```python
from build123d import *

# Parameters (mm, degrees)
SKETCH1_W                                            = 4
SKETCH1_H                                            = 10
BOSS_EXTRUDE1_DEPTH                                  = 18
HOLE_SIZE_SLOTTED_COUNTERSUNK_WOOD_SCREW_D           = 2.4
HOLE_SIZE_SLOTTED_COUNTERSUNK_WOOD_SCREW_CSINK_D     = 4.5
HOLE_SIZE_SLOTTED_COUNTERSUNK_WOOD_SCREW_CSINK_ANGLE = 90
M2_TAPPED_HOLE1_D                                    = 1.6
M2_TAPPED_HOLE1_DEPTH                                = 6.4
M2_TAPPED_HOLE1_TIP                                  = 0.480688495
FILLET1_R                                            = 2.5
CHAMFER1_SIZE                                        = 0.2


with BuildPart() as part:
    # Sketch1 → Boss-Extrude1 (new body)
    with BuildSketch(Plane(origin=(0, 0, 0), x_dir=(1, 0, 0), z_dir=(0, 1, 0))):
        with Locations((2, 5)):
            Rectangle(SKETCH1_W, SKETCH1_H)
    extrude(amount=BOSS_EXTRUDE1_DEPTH)

    # Hole size slotted countersunk wood screw type 1 (through all)
    with Locations(Plane(origin=(4, 0, 0), x_dir=(0, 0, -1), z_dir=(1, 0, 0))):
        with Locations((2.5, 15.5), (7.5, 15.5)):
            CounterSinkHole(HOLE_SIZE_SLOTTED_COUNTERSUNK_WOOD_SCREW_D / 2, HOLE_SIZE_SLOTTED_COUNTERSUNK_WOOD_SCREW_CSINK_D / 2, counter_sink_angle=HOLE_SIZE_SLOTTED_COUNTERSUNK_WOOD_SCREW_CSINK_ANGLE)

    # M2 Tapped Hole1
    with Locations(Plane(origin=(0, 0, 0), x_dir=(-1, 0, 0), z_dir=(0, -1, 0))):
        with Locations((-2, 2.5), (-2, 7.5)):
            Hole(M2_TAPPED_HOLE1_D / 2, depth=M2_TAPPED_HOLE1_DEPTH)
            with Locations((0, 0, -(M2_TAPPED_HOLE1_DEPTH + M2_TAPPED_HOLE1_TIP / 2))):  # 118° drill point
                Cone(0, M2_TAPPED_HOLE1_D / 2, M2_TAPPED_HOLE1_TIP, mode=Mode.SUBTRACT)

    # Fillet1
    fillet1_edges = [part.edges().sort_by_distance(p)[0] for p in [
        (2, 18, -10),
    ]]
    fillet(fillet1_edges, radius=FILLET1_R)

    # Chamfer1
    chamfer1_edges = [part.edges().sort_by_distance(p)[0] for p in [
        (4, 18, -3.75),
        (0, 15.5, -8.7),
        (0, 15.5, -3.7),
        (1.2, 0, -7.5),
        (1.2, 0, -2.5),
        (0, 18, -3.75),
        (0, 7.75, -10),
        (0, 17.267766953, -9.267766953),
        (4, 7.75, -10),
        (4, 17.267766953, -9.267766953),
        (2, 0, -10),
        (4, 0, -5),
        (2, 0, 0),
        (0, 0, -5),
        (4, 9, 0),
        (0, 9, 0),
        (2, 18, 0),
    ]]
    chamfer(chamfer1_edges, length=CHAMFER1_SIZE)


solid = part.part
```
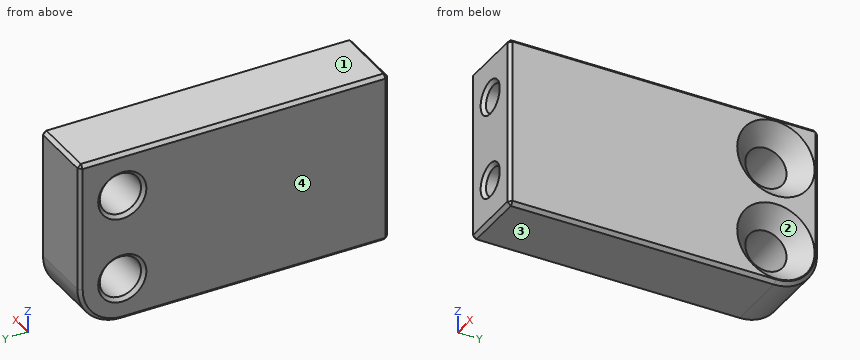
Geometry: final body of the model. Coordinates: model frame, mm. Face numbers are marked on the shaded views. Round coordinates to 2 decimals unless told otherwise and drop trailing zeros. Write each loop counter-clockwise with the first axis right and the second up, starting at its lowest first coordinate (ties: lowest second). Pieces come first, ordered by that corner, then holes.
Item 1: Section query B-B (x = 1.7). Give the number of separate pieces and of enclosed holes in the cut face, plus the area to 3 significant figures.
Item 2: Mould query, pull axis Z, two halves, no side actions, for the marked faces 1, 2, 3 and 4. Classes: +Z half, -Z half, draft (parallel to the pull), parting line (faces both ways), or undercut.
Item 3: Section query A-A (y = 5.5). Return loops of the section in (x, z).
Item 4: Material intervals for L1, parallel to Z at x = 2, y = 2; L2, parallel to Z at x = 1.35, y = 15.5; L3, parallel to X at y = 2.25, z = -2.5, sorted ascending.
Item 5: Pin query (flat end, axial travel): P1, Ø1.9, axis at y = 15.5, z = -7.5, coming from the -X side; P2, Ø1.4, axis at x = 2, z = -2.5, coming from the -Y side; P3, Ø3, axis at y = 15.5, z = -2.5, coming from the +X side. Return the tip coordinate at first contact, or that it passes through.
Completed:
1. separate pieces: 1
1. enclosed holes: 2
1. area: 150 mm2
2. face 1: +Z half
2. face 2: undercut
2. face 3: -Z half
2. face 4: draft
3. outline: (0, -9.8) - (0.2, -10) - (3.8, -10) - (4, -9.8) - (4, -0.2) - (3.8, 0) - (0.2, 0) - (0, -0.2) - close; hole circle Ø1.6 at (2, -7.5); hole circle Ø1.6 at (2, -2.5)
4. L1: z = -10 to -8.3, -6.7 to -3.3, -1.7 to 0
4. L2: z = -10 to -8.7, -6.3 to -3.7, -1.3 to 0
4. L3: x = 0 to 1.2, 2.8 to 4
5. P1: passes through
5. P2: stops at y = 6.46
5. P3: stops at x = 3.25
